```python
from build123d import *

# Parameters (mm, degrees)
BOSS_EXTRUDE1_DEPTH    = 10
SKETCH3_R              = 5
CUT_EXTRUDE2_DEPTH     = 27
SKETCH5_R              = 1.5
CUT_EXTRUDE4_DEPTH     = 10
M4_TAPPED_HOLE1_D      = 3.3
M4_TAPPED_HOLE1_DEPTH  = 10
M4_TAPPED_HOLE1_TIP    = 0.991420021
SKETCH9_R              = 7.5
CUT_EXTRUDE5_DEPTH     = 10
M3_TAPPED_HOLE2_REACH  = 45.296
M3_TAPPED_HOLE2_BORE_R = 1.25
M3_TAPPED_HOLE3_D      = 2.5
M3_TAPPED_HOLE3_DEPTH  = 10
M3_TAPPED_HOLE3_TIP    = 0.751075774


with BuildPart() as part:
    # Sketch1 → Boss-Extrude1 (new, symmetric)
    with BuildSketch(Plane.XY):
        Polygon((-18, -6.74079026), (-26, -6.74079026), (-26, 28.25920974), (26, 28.25920974), (26, -6.74079026), (18, -6.74079026), (18, 16.25920974), (-18, 16.25920974), align=None)
    extrude(amount=BOSS_EXTRUDE1_DEPTH, both=True)

    # Sketch3 → Cut-Extrude2 (cut)
    with BuildSketch(Plane(origin=(0, 28.25920974, 0), x_dir=(1, 0, 0), z_dir=(0, 1, 0))):
        with Locations(Location((0, 0, 0), (0, 0, 180))):
            Circle(SKETCH3_R)
    extrude(amount=-CUT_EXTRUDE2_DEPTH, mode=Mode.SUBTRACT)

    # Sketch5 → Cut-Extrude4 (cut)
    with BuildSketch(Plane.XZ.offset(6.74079026)):
        with Locations((22, 6)):
            Circle(SKETCH5_R)
        with Locations((22, -6)):
            Circle(SKETCH5_R)
        with Locations(Location((-22, -6, 0), (0, 0, 180))):
            Circle(SKETCH5_R)
        with Locations(Location((-22, 6, 0), (0, 0, 180))):
            Circle(SKETCH5_R)
    extrude(amount=-CUT_EXTRUDE4_DEPTH, mode=Mode.SUBTRACT)

    # M4 Tapped Hole1
    with Locations(Plane(origin=(0, -6.74079026, 0), x_dir=(-1, 0, 0), z_dir=(0, -1, 0))):
        with Locations((-22, 6), (-22, -6), (22, 6), (22, -6)):
            Hole(M4_TAPPED_HOLE1_D / 2, depth=M4_TAPPED_HOLE1_DEPTH)
            with Locations((0, 0, -(M4_TAPPED_HOLE1_DEPTH + M4_TAPPED_HOLE1_TIP / 2))):  # 118° drill point
                Cone(0, M4_TAPPED_HOLE1_D / 2, M4_TAPPED_HOLE1_TIP, mode=Mode.SUBTRACT)

    # Sketch9 → Cut-Extrude5 (cut)
    with BuildSketch(Plane.XZ.offset(-16.25920974)):
        Circle(SKETCH9_R)
    extrude(amount=-CUT_EXTRUDE5_DEPTH, mode=Mode.SUBTRACT)

    # M3 Tapped Hole2 bore → M3 Tapped Hole2 (cut, up to next)
    with BuildSketch(Plane.XY.offset(10), mode=Mode.PRIVATE) as m3_tapped_hole2_sk1:
        with Locations((0, 18.75920974)):
            Circle(M3_TAPPED_HOLE2_BORE_R)
    m3_tapped_hole2_tool1 = extrude(m3_tapped_hole2_sk1.sketch, amount=-M3_TAPPED_HOLE2_REACH, mode=Mode.PRIVATE) & part.part
    add(m3_tapped_hole2_tool1.solids().sort_by_distance((0, 18.75921, 10))[0], mode=Mode.SUBTRACT)

    # M3 Tapped Hole3
    with Locations(Plane(origin=(0, 16.25920974, 0), x_dir=(-1, 0, 0), z_dir=(0, -1, 0))):
        with Locations((10, 0), (-10, 0)):
            Hole(M3_TAPPED_HOLE3_D / 2, depth=M3_TAPPED_HOLE3_DEPTH)
            with Locations((0, 0, -(M3_TAPPED_HOLE3_DEPTH + M3_TAPPED_HOLE3_TIP / 2))):  # 118° drill point
                Cone(0, M3_TAPPED_HOLE3_D / 2, M3_TAPPED_HOLE3_TIP, mode=Mode.SUBTRACT)


solid = part.part
```
Verification items for the finished model (mm, model axes). A direction names the side the tool comes from. Give positions to 0.01 mm unless a question says otherwise; leave off trailing zeros. Order: outer loops, then holes, each group sorted by start corner. A loop starts at its lowest first (then second) coordinate and runs counter-clockwise, first axis right, second up. Notation, with made-up numbers: (-30, -10) - (-14, -10) arc R8 ccw to (-14, 5) - close; hole circle Ø4 at (-8, -3.75). An arc over 180 degrees is marked (long way). Answer as CSV lines item,"result". Start each with the question number.
Item 1: Section check D-D, the plane z = 2. Record the boundary of the cut face in (x, y).
Item 2: Section check C-C, the plane y = 5. Record the boundary of the cut face in (x, z).
Item 3: Section check A-A, the plane x = 0. Record the boundary of the cut face in (y, z), plus the area to 4 significant figures.
Item 4: Mould release check, pull along X, two halves, no side actions. Record for faces 1 (the face through (-26, 11, 0)), 2 (the face through (-22, -6.741, 0)), 3 (the face through (-1.63, 21.19, -7.32)), 4 (the face through (9.8, 26.88, 0.08)): released by +X, released by -X, zero draft, split by the parting line, or undercut.
Item 5: Section check B-B, the plane y = 25. Record the boundary of the cut face in (x, z), plus the area to 3 significant figures.
Item 6: Access from +Z, -Z, +X, -X, +Y, -Y to the whole of each face (thin tool, end or side, straight path). Record for faces 5 (the face through (-0.27, 17.54, 8.71)), 6 (the face through (-18, 5, 0)), 7 (the face through (20.35, -1.67, 5.93)), 8 (the face through (0, 23, 10)).
Item 7: Gauge pin test, flat ends, axial feed: pin 1 (12 mm diameter, centred on x = 0, z = 0, fed in from -Y); pin 2 (10 mm diameter, centred on x = -7, z = -2, fed in from -Y); pin 3 (2 mm diameter, centred on x = 22, z = -6, fed in from -Y). Record the tip position at first contact, or that the pin passes through.
Item 8: Material ranges on L1, parallel to Z at x = 22, y = -3; L2, parallel to X at y = 4, z = -1.25; L3, parallel to X at y = 0.5, z = -7, recorded low to high.
Filled in:
1,outline,"(-26, -6.74) - (-18, -6.74) - (-18, 16.26) - (-7.23, 16.26) - (-7.23, 26.26) - (-4.58, 26.26) - (-4.58, 28.26) - (-26, 28.26) - close; (4.58, 26.26) - (7.23, 26.26) - (7.23, 16.26) - (18, 16.26) - (18, -6.74) - (26, -6.74) - (26, 28.26) - (4.58, 28.26) - close"
2,outline,"(-26, -10) - (-18, -10) - (-18, 10) - (-26, 10) - close; (18, -10) - (26, -10) - (26, 10) - (18, 10) - close"
3,outline,"(16.26, -10) - (28.26, -10) - (28.26, -5) - (26.26, -5) - (26.26, -7.5) - (16.26, -7.5) - close; (16.26, 7.5) - (17.51, 7.5) - (17.51, 10) - (16.26, 10) - close; (20.01, 7.5) - (26.26, 7.5) - (26.26, 5) - (28.26, 5) - (28.26, 10) - (20.01, 10) - close"
3,area,"63.75 mm^2"
4,face 1,"released by -X"
4,face 2,"zero draft"
4,face 3,"undercut"
4,face 4,"undercut"
5,outline,"(-26, -10) - (26, -10) - (26, 10) - (-26, 10) - close; hole circle Ø2.5 at (-10, 0); hole circle Ø15 at (0, 0); hole circle Ø2.5 at (10, 0)"
5,area,"853 mm^2"
6,face 5,"+Z"
6,face 6,"+Z, -Z, -Y"
6,face 7,"-Y"
6,face 8,"+Z, +X, -X, +Y, -Y"
7,pin 1,"y = 26.26"
7,pin 2,"y = 16.26"
7,pin 3,"y = 3.65"
8,L1,"-10 to -7.65, -4.35 to 4.35, 7.65 to 10"
8,L2,"-26 to -18, 18 to 26"
8,L3,"-26 to -23.31, -20.69 to -18, 18 to 20.69, 23.31 to 26"
